Verification items for the finished model (mm, model axes). A direction names the side the tool comes from. Give positions to 0.01 mm unless a question says otherwise; leave off trailing zeros. Write each loop counter-clockwise with the first axis right and the second up, starting at its lowest first coordinate (ties: lowest second). Pieces come first, ordered by that corner, then holes. Notation, with made-up numbers: (44.5, 17.25) -> (55.5, 17.25) arc R28 ccw to (55.5, 47.25) -> close; hole circle Ø3 at (81.5, -32.75). An arc over 180 degrees is marked (long way). Use one line per item in the form item = value. Start each with the question number.
(1) Section check B-B, the plane y = 26.5. Record the cut outline in (x, z), plus the area to 3 significant figures.
(2) Section check C-C, the plane z = -10. Record the cut outline in (x, y).
(3) Release check for a two-part mould opening along X. For faces 6 (the face through (11.726, 20.14, -49.3)), 7 (the face through (25, -30, -49)), 8 (the face through (-30, -18, -49)) record: pulls with the +X half, pulls with the -X half, needs draft (parallel to the pull), parting line crosses it, or undercut.
(4) Set-up check for faces 1 (the face through (30, -18, -49)), 2 (the face through (-11.49, 19.86, -49.3)), 3 (the face through (27, 6, -49)), 4 (the face through (0, -10, -49)), 5 (the face through (-27, 6, -49)): record each of +Z, -Z, +X, -X, +Y, -Y from which the full face is reachable in a straight line by a thin tool's end or side.
(5) Section check A-A, the plane x = 25.5. Record the cut outline in (y, z).
(6) Scan lines: L1, parallel to Y at x = 25, z = -74; L2, parallel to X at y = -3.5, z = -11; L3, parallel to X at y = -26.5, z = -31. Record each from-to range of solid material in increasing order.
(7) Depth check by flat-ended pin: pin 1 Ø3 at (x, z) = (-1, -71.5) entering from +Y; pin 2 Ø1 at (x, z) = (0.5, -47.5) entering from -Y; pin 3 Ø3 at (x, z) = (11, -56) entering from +Y. Enter the tip coordinate at first touch or a pass-through.
(8) Section check D-D, the plane x = -1. Record the cut outline in (y, z), plus the area to 3 significant figures.
from build123d import *

# Parameters (mm, degrees)
V_BLOCK_BODY_EXTRUDE_100_DEPTH = 100


with BuildPart() as part:
    # V-Block Profile Sketch → V-Block Body Extrude 100 (new body)
    with BuildSketch(Plane.XY):
        Polygon((-30, -6), (-30, -30), (-20, -30), (-3.218007376, -10), (0, -10), (3.218007376, -10), (20, -30), (30, -30), (30, -6), (24, -6), (24, 6), (30, 6), (30, 30), (20, 30), (3.218007376, 10), (0, 10), (-3.218007376, 10), (-20, 30), (-30, 30), (-30, 6), (-24, 6), (-24, -6), align=None)
    extrude(amount=-V_BLOCK_BODY_EXTRUDE_100_DEPTH)


solid = part.part
Completed:
q1.outline = (-30, -100) -> (-17.06, -100) -> (-17.06, 0) -> (-30, 0) -> close; (17.06, -100) -> (30, -100) -> (30, 0) -> (17.06, 0) -> close
q1.area = 2,590 mm²
q2.outline = (-30, -30) -> (-20, -30) -> (-3.22, -10) -> (3.22, -10) -> (20, -30) -> (30, -30) -> (30, -6) -> (24, -6) -> (24, 6) -> (30, 6) -> (30, 30) -> (20, 30) -> (3.22, 10) -> (-3.22, 10) -> (-20, 30) -> (-30, 30) -> (-30, 6) -> (-24, 6) -> (-24, -6) -> (-30, -6) -> close
q3.face_6 = undercut
q3.face_7 = needs draft
q3.face_8 = pulls with the -X half
q4.face_1 = +Z, -Z, +X, +Y, -Y
q4.face_2 = +Z, -Z, +Y
q4.face_3 = +Z, -Z, +X
q4.face_4 = +Z, -Z, -Y
q4.face_5 = +Z, -Z, -X
q5.outline = (-30, -100) -> (-6, -100) -> (-6, 0) -> (-30, 0) -> close; (6, -100) -> (30, -100) -> (30, 0) -> (6, 0) -> close
q6.L1 = -30 to -6, 6 to 30
q6.L2 = -24 to 24
q6.L3 = -30 to -17.06, 17.06 to 30
q7.pin_1 = 10
q7.pin_2 = -10
q7.pin_3 = 21.06
q8.outline = (-10, -100) -> (10, -100) -> (10, 0) -> (-10, 0) -> close
q8.area = 2,000 mm²
